```python
from build123d import *

# Parameters (mm, degrees)
EXTRUDE_1_DEPTH     = 500
CUT_EXTRUDE_1_DEPTH = 480


with BuildPart() as part:
    # 草图1 → 凸台-拉伸1 (new body)
    with BuildSketch(Plane.XY):
        with BuildLine():
            Line((-46.8, 25), (46.8, 25))
            ThreePointArc((46.8, 25), (49.0627417, 24.0627417), (50, 21.8))
            Line((50, 21.8), (50, -21.8))
            ThreePointArc((50, -21.8), (49.0627417, -24.0627417), (46.8, -25))
            Line((46.8, -25), (-46.8, -25))
            ThreePointArc((-46.8, -25), (-49.0627417, -24.0627417), (-50, -21.8))
            Line((-50, -21.8), (-50, 21.8))
            ThreePointArc((-50, 21.8), (-49.0627417, 24.0627417), (-46.8, 25))
        make_face()
        with BuildLine():
            Line((-46.8, 22), (46.8, 22))
            ThreePointArc((46.8, 22), (46.941421356, 21.941421356), (47, 21.8))
            Line((47, 21.8), (47, -21.8))
            ThreePointArc((47, -21.8), (46.941421356, -21.941421356), (46.8, -22))
            Line((46.8, -22), (-46.8, -22))
            ThreePointArc((-46.8, -22), (-46.941421356, -21.941421356), (-47, -21.8))
            Line((-47, -21.8), (-47, 21.8))
            ThreePointArc((-47, 21.8), (-46.941421356, 21.941421356), (-46.8, 22))
        make_face(mode=Mode.SUBTRACT)
    extrude(amount=EXTRUDE_1_DEPTH)

    # 草图3 → 切除-拉伸1 (cut)
    with BuildSketch(Plane(origin=(50, 0, 0), x_dir=(0, 0, -1), z_dir=(1, 0, 0))):
        Polygon((-70, 25), (-20, -25), (18.010342751, -26.423264748), (18.010342751, 25), align=None)
    extrude(amount=-CUT_EXTRUDE_1_DEPTH, mode=Mode.SUBTRACT)


solid = part.part
```
Work out the finished part from the listing and answer in its coordinate system (mm). A direction names the side the tool comes from. Round coordinates to 2 decimals unless told otherwise and drop trailing zeros. Write each loop counter-clockwise with the first axis right and the second up, starting at its lowest first coordinate (ties: lowest second). Pieces come first, ordered by that corner, then holes.
1) A cutting plane is placed at A-A on y = 5. Determine the outline of the cut face in (x, z), and give its area (3 significant figures).
2) Determine the mould class of faces 1 (the face through (-1, 22, 280)), 2 (the face through (50, 0, 258)), 3 (the face through (0, -24, 500)) for opening direction X: pulls with the +X half, pulls with the -X half, needs draft (parallel to the pull), parting line crosses it, or undercut.
3) Consider probe 1 along X at (y, z) = (-2, 233); probe 2 along Y at (x, z) = (-40, 456); probe 3 along X at (y, z) = (-23, 101.5). Determine where each line is inside the solid, lowest interval first.
4) A cutting plane is placed at C-C on x = 37. Determine the outline of the cut face in (y, z), and give its area (3 significant figures).
5) A cutting plane is placed at B-B on z = 234. Determine the outline of the cut face in (x, y), and give its area (3 significant figures).
6) A cutting plane is placed at D-D on z = 55.5. Determine the outline of the cut face in (x, y), and give its area (3 significant figures).
7) Which of the six approach directions +Z, -Z, +X, -X, +Y, -Y give full straight-line access (tool end or side, diameter ignored) to faces 4 (the face through (1, -25, 257)), 5 (the face through (-47, 0, 258))?
Entries:
1. outline: (-50, 50) - (-47, 50) - (-47, 500) - (-50, 500) - close; (47, 50) - (50, 50) - (50, 500) - (47, 500) - close
1. area: 2,700 mm2
2. face 1: undercut
2. face 2: pulls with the +X half
2. face 3: needs draft
3. probe 1: x = -50 to -47, 47 to 50
3. probe 2: y = -25 to -22, 22 to 25
3. probe 3: x = -49.77 to 49.77
4. outline: (-25, 20) - (-22, 23) - (-22, 500) - (-25, 500) - close; (22, 67) - (25, 70) - (25, 500) - (22, 500) - close
4. area: 2,730 mm2
5. outline: (-50, -21.8) arc R3.2 ccw to (-46.8, -25) - (46.8, -25) arc R3.2 ccw to (50, -21.8) - (50, 21.8) arc R3.2 ccw to (46.8, 25) - (-46.8, 25) arc R3.2 ccw to (-50, 21.8) - close; hole (-47, -21.8) arc R0.2 ccw to (-46.8, -22) - (46.8, -22) arc R0.2 ccw to (47, -21.8) - (47, 21.8) arc R0.2 ccw to (46.8, 22) - (-46.8, 22) arc R0.2 ccw to (-47, 21.8) - close
5. area: 855 mm2
6. outline: (-50, -21.8) arc R3.2 ccw to (-46.8, -25) - (46.8, -25) arc R3.2 ccw to (50, -21.8) - (50, 10.5) - (47, 10.5) - (47, -21.8) arc R0.2 cw to (46.8, -22) - (-46.8, -22) arc R0.2 cw to (-47, -21.8) - (-47, 10.5) - (-50, 10.5) - close
6. area: 491 mm2
7. face 4: +Z, -Z, +X, -X, -Y
7. face 5: +Z, -Z
